```python
from build123d import *

# Parameters (mm, degrees)
BOSS_EXTRUDE1_DEPTH = 28


with BuildPart() as part:
    # Sketch1 → Boss-Extrude1 (new body)
    with BuildSketch(Plane(origin=(0, 0, 0), x_dir=(1, 0, 0), z_dir=(0, 1, 0))):
        Polygon((2750.872583656, 1604.162796977), (3065.872583656, 1604.162796977), (3080.872583656, 1619.162796977), (3080.872583656, 1664.162796977), (2750.872583656, 1624.162796977), align=None)
    extrude(amount=BOSS_EXTRUDE1_DEPTH)


solid = part.part
```
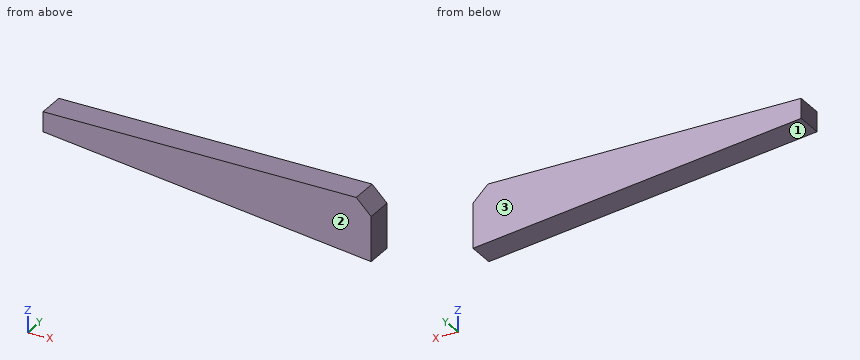
Design review of the part built by this model. Coordinates are the model's own, in mm. Face numbers are marked on the shaded views. Coordinates: 2 decimals unless noted, no trailing zeros. Order: outer loops, then holes, each group sorted by start corner. A loop starts at its lowest first (then second) coordinate and runs counter-clockwise, first axis right, second up.
1) Mouldability with a two-part tool opening along Y and no side actions: class the marked faces 1, 2 and 3 as +Y half, -Y half, draft (parallel to the pull), parting line (faces both ways), or undercut.
2) Take a section at B-B, the plane x = 2842.5. Give the boundary of the cut face in (y, z), and give its area (3 significant figures).
3) Take a section at A-A, the plane y = 24. Give the boundary of the cut face in (x, z), and give its area (3 significant figures).
4) Clearance check with a flat-ended pin moving along its axis: pin 1 (3 mm diameter, centred on x = 2806, y = 7.5, fed in from -Z). State where the tip first meets the part, or that it passes through.
5) Wall thickness on line 1 along Z through (x, y) = (2973.5, 2.75); line 2 along Z through (x, y) = (2952.5, 8); line 3 along X through (y, z) = (8, -1613): over which ranges is each line inside the solid? List them lowest first.
6) Take a section at C-C, the plane z = -1608. Give the boundary of the cut face in (x, y).
Returned:
1. face 1: draft
1. face 2: -Y half
1. face 3: +Y half
2. outline: (0, -1635.27) - (28, -1635.27) - (28, -1604.16) - (0, -1604.16) - close
2. area: 871 mm2
3. outline: (2750.87, -1624.16) - (3080.87, -1664.16) - (3080.87, -1619.16) - (3065.87, -1604.16) - (2750.87, -1604.16) - close
3. area: 13,100 mm2
4. pin 1: stops at z = -1631.03
5. line 1: z = -1651.15 to -1604.16
5. line 2: z = -1648.6 to -1604.16
5. line 3: x = 2750.87 to 3074.71
6. outline: (2750.87, 0) - (3069.71, 0) - (3069.71, 28) - (2750.87, 28) - close
